Here's how the part is built. I have some questions about the finished solid (model axes, mm). A direction names the side the tool comes from. Coordinates: 2 decimals unless noted, no trailing zeros. Order: outer loops, then holes, each group sorted by start corner. A loop starts at its lowest first (then second) coordinate and runs counter-clockwise, first axis right, second up. Notation, with made-up numbers: (5.5, 88.25) - (23.5, 88.25) arc R22 cw to (23.5, 110.25) - close; hole circle Ø3 at (36.5, 18). An arc over 180 degrees is marked (long way). Answer as CSV lines item,"result". Start each with the question number.
Q1. I need wall thicknesses on line 1 (Y direction, x = 0, z = -12.5); line 2 (Y direction, x = 2.5, z = -5.5); line 3 (X direction, y = 0.3, z = -4.5). Which ranges of each line are inside material? Lowest first, please.
Q2. For faces 1 (the face through (1, 1, -8.333)), 2 (the face through (6, 0, -12)), which set-ups out of +Z, -Z, +X, -X, +Y, -Y let a thin tool reach every point of the face, with its end or its side?
Q3. Suppose I cut it at D-D (y = 0.55). Please give me the cut outline in (x, z), then the cut area to 3 significant figures.
Q4. Thinking about a two-plate mould opening in X: for faces 3 (the face through (5.35, 0.39, -18.93)), 4 (the face through (1, 1, -16.667)), which applies, released by +X, released by -X, zero draft, split by the parting line, or undercut?
Q5. Suppose I cut it at B-B (y = 1.9). Please give me the cut outline in (x, z), then the cut area to 3 significant figures.
Q6. For pin 1 Ø2.5 at (x, z) = (6, -4.5) entering from +Y; pin 2 Ø1.5 at (y, z) = (0.5, -12.5) entering from -X; pin 3 Ø7 at (x, z) = (6.5, -7.5) entering from +Y; pin 4 Ø0.6 at (y, z) = (0.5, -20) entering from -X, each with a flat end and sliding along its axis, tell me the tip position at first contact or that it passes through.
Q7. Suppose I cut it at A-A (x = 6). Please give me the cut outline in (y, z).
Q8. Suppose I cut it at C-C (z = -4.5). Please give me the cut outline in (x, y), then the cut area to 3 significant figures.
from build123d import *

# Parameters (mm, degrees)
SKETCH_1_R          = 1
EXTRUDE_1_DEPTH     = 25
CUT_EXTRUDE_1_DEPTH = 3.8
SKETCH_3_R          = 1.7
CUT_EXTRUDE_2_DEPTH = 0.8
SKETCH_4_R          = 1.7
CUT_EXTRUDE_3_DEPTH = 0.8


with BuildPart() as part:
    # 草图1 → 凸台-拉伸1 (new body)
    with BuildSketch(Plane.XY):
        with BuildLine():
            Line((0, 0), (10, 0))
            Line((10, 0), (10, 0.8))
            Line((10, 0.8), (1.549193338, 0.8))
            ThreePointArc((1.549193338, 0.8), (-0.871779789, 3.588194302), (0, 0))
        make_face()
        with Locations((0, 1.9)):
            Circle(SKETCH_1_R, mode=Mode.SUBTRACT)
    extrude(amount=-EXTRUDE_1_DEPTH)

    # 草图2 → 切除-拉伸1 (cut)
    with BuildSketch(Plane(origin=(0, 0, 0), x_dir=(1, 0, 0), z_dir=(0, 1, 0))):
        Polygon((-6, 0), (2.09, 0), (2.09, 8.333333333), (-2.09, 8.333333333), (-2.09, 16.666666667), (2.09, 16.666666667), (2.09, 25), (-6, 25), align=None)
    extrude(amount=CUT_EXTRUDE_1_DEPTH, mode=Mode.SUBTRACT)

    # 草图3 → 切除-拉伸2 (cut)
    with BuildSketch(Plane(origin=(0, 0, 0), x_dir=(1, 0, 0), z_dir=(0, 1, 0))):
        with Locations(Location((6, 20.5, 0), (0, 0, 270))):
            Circle(SKETCH_3_R)
    extrude(amount=CUT_EXTRUDE_2_DEPTH, mode=Mode.SUBTRACT)

    # 草图4 → 切除-拉伸3 (cut)
    with BuildSketch(Plane(origin=(0, 0, 0), x_dir=(1, 0, 0), z_dir=(0, 1, 0))):
        with Locations(Location((6, 4.5, 0), (0, 0, 270))):
            Circle(SKETCH_4_R)
    extrude(amount=CUT_EXTRUDE_3_DEPTH, mode=Mode.SUBTRACT)


solid = part.part
Here are the results:
1,line 1,"y = 0 to 0.9, 2.9 to 3.8"
1,line 2,"y = 0 to 0.8"
1,line 3,"x = 2.09 to 4.3, 7.7 to 10"
2,face 1,"+Z, -X, +Y, -Y"
2,face 2,"+Z, -Z, +X, -X, -Y"
3,outline,"(-1.34, -16.67) - (2.09, -16.67) - (2.09, -25) - (10, -25) - (10, 0) - (2.09, 0) - (2.09, -8.33) - (-1.34, -8.33) - close; hole circle Ø3.4 at (6, -20.5); hole circle Ø3.4 at (6, -4.5)"
3,area,"208 mm²"
4,face 3,"undercut"
4,face 4,"zero draft"
5,outline,"(-1.9, -16.67) - (-1, -16.67) - (-1, -8.33) - (-1.9, -8.33) - close; (1, -16.67) - (1.9, -16.67) - (1.9, -8.33) - (1, -8.33) - close"
5,area,"15.0 mm²"
6,pin 1,"passes through"
6,pin 2,"stops at x = -1.79"
6,pin 3,"stops at y = 0.8"
6,pin 4,"stops at x = 2.09"
7,outline,"(0, -25) - (0.8, -25) - (0.8, -22.2) - (0, -22.2) - close; (0, -18.8) - (0.8, -18.8) - (0.8, -6.2) - (0, -6.2) - close; (0, -2.8) - (0.8, -2.8) - (0.8, 0) - (0, 0) - close"
8,outline,"(2.09, 0) - (4.3, 0) - (4.3, 0.8) - (2.09, 0.8) - close; (7.7, 0) - (10, 0) - (10, 0.8) - (7.7, 0.8) - close"
8,area,"3.61 mm²"
